```python
from build123d import *

# Parameters (mm, degrees)
L_BRACKET_PROFILE_SKETCH_W     = 140
L_BRACKET_PROFILE_SKETCH_H     = 76
L_BRACKET_BASE_DEPTH           = 28
STEPPED_BLOCK_CUT_DEPTH        = 36
RECTANGULAR_POCKET_SKETCH_W    = 30
RECTANGULAR_POCKET_SKETCH_H    = 22
RECTANGULAR_POCKET_30X22_DEPTH = 10
UPRIGHT_RECESS_SKETCH_W        = 38
UPRIGHT_RECESS_SKETCH_H        = 56
UPRIGHT_FACE_RECESS_DEPTH      = 6
UPRIGHT_SLOT_AND_HOLE_SKETCH_R = 9
UPRIGHT_SLOT_AND_HOLE_DEPTH    = 88.407093534
CORNER_NOTCH_DEPTH             = 20
HORIZONTAL_SLOT_9_5_WIDE_DEPTH = 115.210332282
POCKET_HOLE_SKETCH_R           = 6
POCKET_HOLE_12_DEPTH           = 20
EDGE_FILLETS_R5_R              = 5


with BuildPart() as part:
    # L-Bracket Profile Sketch → L-Bracket Base (new, symmetric)
    with BuildSketch(Plane.XY):
        Rectangle(L_BRACKET_PROFILE_SKETCH_W, L_BRACKET_PROFILE_SKETCH_H)
    extrude(amount=L_BRACKET_BASE_DEPTH, both=True)

    # Step Cut Sketch → Stepped Block Cut (cut)
    with BuildSketch(Plane.XY.offset(28)):
        Polygon((-70, 8), (-34, 8), (-34, -18), (70, -18), (70, 38), (-70, 38), align=None)
    extrude(amount=-STEPPED_BLOCK_CUT_DEPTH, mode=Mode.SUBTRACT)

    # Rectangular Pocket Sketch → Rectangular Pocket 30x22 (cut)
    with BuildSketch(Plane(origin=(0, -18, 0), x_dir=(1, 0, 0), z_dir=(0, 1, 0))):
        with Locations((-4, -17)):
            Rectangle(RECTANGULAR_POCKET_SKETCH_W, RECTANGULAR_POCKET_SKETCH_H)
    extrude(amount=-RECTANGULAR_POCKET_30X22_DEPTH, mode=Mode.SUBTRACT)

    # Upright Recess Sketch → Upright Face Recess (cut)
    with BuildSketch(Plane.XY.offset(-8)):
        with Locations((51, 10)):
            Rectangle(UPRIGHT_RECESS_SKETCH_W, UPRIGHT_RECESS_SKETCH_H)
    extrude(amount=-UPRIGHT_FACE_RECESS_DEPTH, mode=Mode.SUBTRACT)

    # Upright Slot and Hole Sketch → Upright Slot and Hole (cut, through all)
    with BuildSketch(Plane.XY.offset(-8)):
        with Locations((2, 21)):
            Circle(UPRIGHT_SLOT_AND_HOLE_SKETCH_R)
        with BuildLine():
            Line((45, -4), (45, 26))
            ThreePointArc((45, 26), (51, 32), (57, 26))
            Line((57, 26), (57, -4))
            ThreePointArc((57, -4), (51, -10), (45, -4))
        make_face()
    extrude(amount=-UPRIGHT_SLOT_AND_HOLE_DEPTH, mode=Mode.SUBTRACT)

    # Corner Notch Sketch → Corner Notch (cut)
    with BuildSketch(Plane(origin=(0, 38, 0), x_dir=(1, 0, 0), z_dir=(0, 1, 0))):
        Polygon((-70, 13), (-65, 8), (-70, 8), align=None)
        with BuildLine():
            Line((-70, 23), (-70, 28))
            Line((-70, 28), (-65, 28))
            ThreePointArc((-65, 28), (-68.535533906, 26.535533906), (-70, 23))
        make_face()
    extrude(amount=-CORNER_NOTCH_DEPTH, mode=Mode.SUBTRACT)

    # Horizontal Slot Sketch → Horizontal Slot 9.5 Wide (cut, through all)
    with BuildSketch(Plane(origin=(-34, 0, 0), x_dir=(0, 0, -1), z_dir=(1, 0, 0))):
        with BuildLine():
            Line((-18.5, 1), (-1.5, 1))
            ThreePointArc((-1.5, 1), (4.5, -5), (-1.5, -11))
            Line((-1.5, -11), (-18.5, -11))
            ThreePointArc((-18.5, -11), (-24.5, -5), (-18.5, 1))
        make_face()
    extrude(amount=-HORIZONTAL_SLOT_9_5_WIDE_DEPTH, mode=Mode.SUBTRACT)

    # Pocket Hole Sketch → Pocket Hole Ø12 (cut)
    with BuildSketch(Plane(origin=(0, -28, 0), x_dir=(1, 0, 0), z_dir=(0, 1, 0))):
        with Locations(Location((-4, -17, 0), (0, 0, 270))):
            Circle(POCKET_HOLE_SKETCH_R)
    extrude(amount=-POCKET_HOLE_12_DEPTH, mode=Mode.SUBTRACT)

    # Edge Fillets R5
    edge_fillets_r5_edges = [part.edges().sort_by_distance(p)[0] for p in [
        (70, -28, 28),
        (70, 38, -21),
    ]]
    fillet(edge_fillets_r5_edges, radius=EDGE_FILLETS_R5_R)


solid = part.part
```
Geometry: final body of the model. Coordinates: model frame, mm. A direction names the side the tool comes from. Give positions to 0.01 mm unless a question says otherwise; leave off trailing zeros. Loops run counter-clockwise (first coordinate to the right, second up) from the corner with the lowest first, then second, coordinate; pieces in that order, holes last. Notation, with made-up numbers: (43.5, 12) -> (66.5, 12) arc R10 cw to (66.5, 19) -> close; hole circle Ø7 at (28.25, 41.25). An arc over 180 degrees is marked (long way). Use CSV: the item, a comma, the result in double quotes.
(1) Cut plane C-C (z = -20). Output: boundary loops of the cut face in (x, y), plus the area to 3 significant figures.
From the geometry:
outline,"(-70, -38) -> (70, -38) -> (70, 33) arc R5 ccw to (65, 38) -> (-70, 38) -> close; hole circle Ø18 at (2, 21); hole (45, -4) arc R6 ccw to (57, -4) -> (57, 26) arc R6 ccw to (45, 26) -> close"
area,"9,910 mm^2"
(2) First-contact query: P1, Ø3, axis at x = -8, y = -25, coming from the +Z side; P2, Ø1.5, axis at x = 6, y = -17, coming from the +Z side; P3, Ø11, axis at x = 2, y = 21, coming from the +Z side; P4, Ø14, axis at x = -4, z = 17, coming from the +Y side. Flat tips, straight axial feed; report the tip coordinate or a pass-through.
From the geometry:
P1,"z = 6"
P2,"z = -8"
P3,"through"
P4,"y = -28"
(3) Access query for faces 5 (the face through (-68, 28, -11)), 6 (the face through (11, -23, 17)), 7 (the face through (32, 10, -11)), 8 (the face through (51, -10, -21)), 9 (the face through (-52, 8, 10)). Directions: +Z, -Z, +X, -X, +Y, -Y. A direction counts if a zero-diameter tool reaches every point of the face in a straight line with its end or side. Return the directions, or none.
From the geometry:
face 5,"+Z, -X, +Y"
face 6,"+Z, +Y"
face 7,"+Z, +X, +Y"
face 8,"+Z, -Z"
face 9,"+Z, +X, -X, +Y"
(4) Cut plane B-B (x = -54). Output: boundary loops of the cut face in (y, z).
From the geometry:
outline,"(-38, -28) -> (38, -28) -> (38, -8) -> (8, -8) -> (8, 28) -> (-38, 28) -> close; hole (-11, 1.5) arc R6 ccw to (1, 1.5) -> (1, 18.5) arc R6 ccw to (-11, 18.5) -> close"
(5) Ray query, line 1 along X through (y, z) = (-25, 13.5); line 2 along X through (y, z) = (-35, 17); line 3 along Y through (x, z) = (2, -23.5). Return the intervals inside material, ascending. Write a range as [from, to].
From the geometry:
line 1,"[-70, -19], [11, 70]"
line 2,"[-70, -10], [2, 70]"
line 3,"[-38, 12], [30, 38]"
(6) Cut plane A-A (z = 17). Output: boundary loops of the cut face in (x, y), plus the area to 3 significant figures.
From the geometry:
outline,"(-70, -38) -> (-10, -38) -> (-10, -28) -> (-19, -28) -> (-19, -18) -> (-34, -18) -> (-34, -11) -> (-70, -11) -> close; (-70, 1) -> (-34, 1) -> (-34, 8) -> (-70, 8) -> close; (2, -38) -> (70, -38) -> (70, -18) -> (11, -18) -> (11, -28) -> (2, -28) -> close"
area,"2,880 mm^2"
(7) Pull-direction query (Z, two-part tool) for faces 1 (the face through (-52, -11, 10)), 2 (the face through (-68, 28, -27)), 3 (the face through (-52, 1, 10)), 4 (the face through (-34, 4, 10)); classes: released by +Z, released by -Z, zero draft, split by the parting line, or undercut.
From the geometry:
face 1,"undercut"
face 2,"released by -Z"
face 3,"undercut"
face 4,"zero draft"
(8) Cut plane D-D (x = 53). Output: boundary loops of the cut face in (y, z).
From the geometry:
outline,"(-38, -28) -> (-9.66, -28) -> (-9.66, -14) -> (-18, -14) -> (-18, 28) -> (-38, 28) -> close; (31.66, -28) -> (38, -28) -> (38, -14) -> (31.66, -14) -> close"
